```python
from build123d import *

# Parameters (mm, degrees)
SKETCH2_R           = 3.81
BOSS_EXTRUDE1_DEPTH = 8.382
SKETCH3_W           = 6.35
SKETCH3_H           = 2.159
CUT_EXTRUDE3_DEPTH  = 35.847818067
SKETCH4_R           = 6.35
CUT_EXTRUDE5_DEPTH  = 2.159
CUT_EXTRUDE6_START  = -2.159
SKETCH5_R           = 6.35
CUT_EXTRUDE6_DEPTH  = 2.159
SCALE1_SCALE        = 2


with BuildPart() as part:
    # Sketch2 → Boss-Extrude1 (new body)
    with BuildSketch(Plane(origin=(0, 0, 0), x_dir=(1, 0, 0), z_dir=(0, 1, 0))):
        with BuildLine():
            Line((0, 6.35), (25, 6.35))
            ThreePointArc((25, 6.35), (31.35, 0), (25, -6.35))
            Line((25, -6.35), (0, -6.35))
            ThreePointArc((0, -6.35), (-6.35, 0), (0, 6.35))
        make_face()
        with Locations(Location((0, 0, 0), (0, 0, 270))):
            Circle(SKETCH2_R, mode=Mode.SUBTRACT)
        with Locations(Location((25, 0, 0), (0, 0, 270))):
            Circle(SKETCH2_R, mode=Mode.SUBTRACT)
    extrude(amount=BOSS_EXTRUDE1_DEPTH)

    # Sketch3 → Cut-Extrude3 (cut, through all)
    with BuildSketch(Plane.XY.offset(6.35)):
        Polygon((52.142468872, 2.159), (25, 2.159), (25, 0), (54.039711746, 0), align=None)
        with Locations((21.825, 1.0795)):
            Rectangle(SKETCH3_W, SKETCH3_H)
        Polygon((49.831282098, 8.382), (25, 8.382), (25, 6.223), (51.556048347, 6.223), align=None)
        with Locations((21.825, 7.3025)):
            Rectangle(SKETCH3_W, SKETCH3_H)
    extrude(amount=-CUT_EXTRUDE3_DEPTH, mode=Mode.SUBTRACT)

    # Sketch4 → Cut-Extrude5 (cut)
    with BuildSketch(Plane.XZ):
        with Locations((18.65, 0)):
            Circle(SKETCH4_R)
    extrude(amount=-CUT_EXTRUDE5_DEPTH, mode=Mode.SUBTRACT)

    # Sketch5 → Cut-Extrude6 (cut)
    with BuildSketch(Plane(origin=(0, 8.382, 0), x_dir=(1, 0, 0), z_dir=(0, 1, 0)).offset(CUT_EXTRUDE6_START)):
        with Locations((18.65, 0)):
            Circle(SKETCH5_R)
    extrude(amount=CUT_EXTRUDE6_DEPTH, mode=Mode.SUBTRACT)


with BuildPart() as part_1:
    # Scale1: scaled about (0, 0, 0)
    add(part.part.scale(SCALE1_SCALE))


solid = part_1.part
```
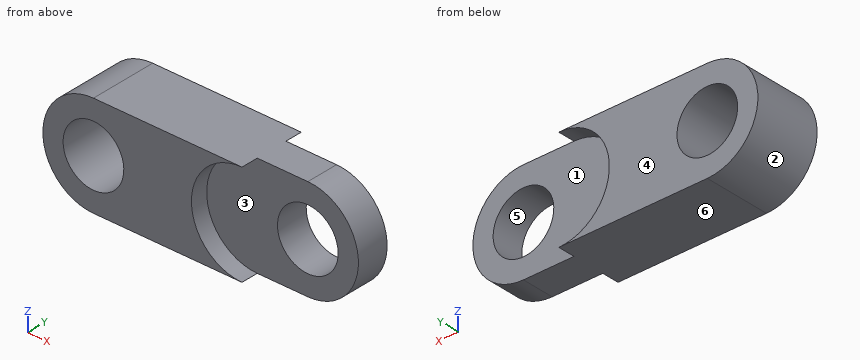
Geometry check sheet. Reference: the model listing, model coordinates, mm. Face numbers are marked on the shaded views. A direction names the side the tool comes from. Coordinates: 2 decimals unless noted, no trailing zeros. Order: outer loops, then holes, each group sorted by start corner. A loop starts at its lowest first (then second) coordinate and runs counter-clockwise, first axis right, second up.
Item 1: Section check B-B (z = 3). Enter the section's corners in (x, y), plus the area to 3 significant figures.
Item 2: Section check D-D (y = 14). Enter the section's corners in (x, z).
Item 3: Scan lines: line 1 along X through (y, z) = (8.75, 0); line 2 along Z through (x, y) = (50, 10); line 3 along X through (y, z) = (13, 0). Record each from-to range of solid material in increasing order.
Item 4: Depth check by flat-ended pin: pin 1 (2 mm diameter, centred on y = 10, z = 5.5, fed in from -X); pin 2 (12.5 mm diameter, centred on x = 38, z = 4.5, fed in from +Y); pin 3 (5 mm diameter, centred on x = -3, z = -2, fed in from -Y); pin 4 (4 mm diameter, centred on y = 13, z = -9, fed in from -X). Enter the tip coordinate at first touch or a pass-through.
Item 5: Mould release check, pull along Z, two halves, no side actions. Record for the marked faces 4, 5 and 6: released by +Z, released by -Z, zero draft, split by the parting line, or undercut.
Item 6: Section check C-C (x = 3). Enter the section's corners in (y, z), plus the area to 3 significant figures.
Item 7: Tool access check on the marked faces 1, 2 and 3. Record the directions out of +Z, -Z, +X, -X, +Y, -Y that give a thin tool (end or side, any length) a straight path to the whole face; none if there is none.
Item 8: Section check A-A (y = 7.75). Enter the section's corners in (x, z).
Check sheet entries:
1. outline: (-12.34, 0) - (-7, 0) - (-7, 16.76) - (-12.34, 16.76) - close; (7, 0) - (24.96, 0) - (24.96, 4.32) - (43, 4.32) - (43, 12.45) - (24.96, 12.45) - (24.96, 16.76) - (7, 16.76) - close; (57, 4.32) - (62.34, 4.32) - (62.34, 12.45) - (57, 12.45) - close
1. area: 580 mm2
2. outline: (0, -12.7) - (37.3, -12.7) arc R12.7 cw to (37.3, 12.7) - (0, 12.7) arc R12.7 ccw to start; hole circle Ø15.24 at (0, 0)
3. line 1: x = -12.7 to -7.62, 7.62 to 42.38, 57.62 to 62.7
3. line 2: z = -12.7 to -7.62, 7.62 to 12.7
3. line 3: x = -12.7 to -7.62, 7.62 to 24.6
4. pin 1: stops at x = -11.88
4. pin 2: stops at y = 12.45
4. pin 3: passes through
4. pin 4: stops at x = -10.6
5. face 4: zero draft
5. face 5: undercut
5. face 6: released by -Z
6. outline: (0, -12.7) - (16.76, -12.7) - (16.76, -7) - (0, -7) - close; (0, 7) - (16.76, 7) - (16.76, 12.7) - (0, 12.7) - close
6. area: 191 mm2
7. face 1: +X, +Y
7. face 2: -X, +Y, -Y
7. face 3: +X, -Y
8. outline: (0, -12.7) - (50, -12.7) arc R12.7 ccw to (50, 12.7) - (0, 12.7) arc R12.7 ccw to start; hole circle Ø15.24 at (0, 0); hole circle Ø15.24 at (50, 0)
